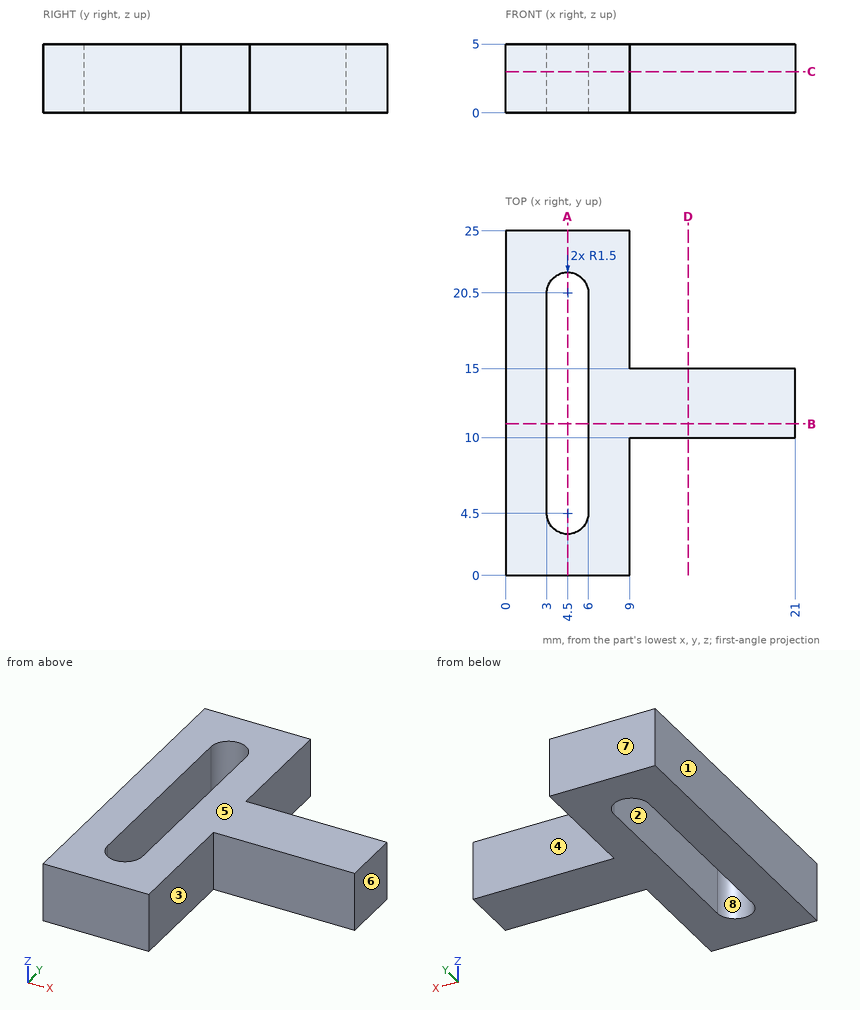
Input: dimensioned drawing with shaded views. Units: mm. Origin: part minimum x, y, z. A direction names the side the tool comes from. Coordinates: 2 decimals unless noted, no trailing zeros. Write each loop counter-clockwise with the first axis right and the second up, starting at its lowest first coordinate (ties: lowest second). Pieces come first, ordered by that corner, then holes. Notation, with made-up numbers: (-14.75, 23) -> (40.25, 23) arc R23 cw to (40.25, 44) -> close; hole circle Ø7 at (-39.5, 81). An arc over 180 degrees is marked (long way). Return JSON: item names as keys, results as strings. Group by question number.
1) Ray query, line 1 along X through (y, z) = (7.5, 1.1); line 2 along X through (y, z) = (12.5, 4.8); line 3 along Y through (x, z) = (10.75, 3.3). Return the intervals inside material, ascending.
2) Section query D-D, the plane x = 13.25. Return loops of the section in (y, z).
3) Section query C-C, the plane z = 3. Return loops of the section in (x, y).
4) Mould query, pull axis X, two halves, no side actions, for the marked faces 6, 7 and 8. Classes: +X half, -X half, draft (parallel to the pull), parting line (faces both ways), or undercut.
5) Section query B-B, the plane y = 11. Return loops of the section in (x, z).
6) Contact query for flat-ended pins moving along their axis: P1, Ø12, axis at x = 12, y = 20, coming from the -Z side; P2, Ø2.5, axis at x = 13.5, z = 3.5, coming from the -Y side; P3, Ø3, axis at x = 16.5, z = 1.5, coming from the +Y side; P4, Ø8, axis at x = 16, y = 20, coming from the -Z side. Output: stop coordinate, or through.
7) Section query A-A, the plane x = 4.5. Return loops of the section in (y, z), plus the area to 3 significant figures.
8) Set-up query: the marked faces 1, 2, 3, 4 and 5. Return all of +Z, -Z, +X, -X, +Y, -Y with unobstructed straight access to the full face (end or side cutting, diameter ignored); none if empty.
From the geometry:
{
 "1": {"line 1": "0 to 3, 6 to 9", "line 2": "0 to 3, 6 to 21", "line 3": "10 to 15"},
 "2": {"outline": "(10, 0) -> (15, 0) -> (15, 5) -> (10, 5) -> close"},
 "3": {"outline": "(0, 0) -> (9, 0) -> (9, 10) -> (21, 10) -> (21, 15) -> (9, 15) -> (9, 25) -> (0, 25) -> close; hole (3, 4.5) arc R1.5 ccw to (6, 4.5) -> (6, 20.5) arc R1.5 ccw to (3, 20.5) -> close"},
 "4": {"face 6": "+X half", "face 7": "draft", "face 8": "undercut"},
 "5": {"outline": "(0, 0) -> (3, 0) -> (3, 5) -> (0, 5) -> close; (6, 0) -> (21, 0) -> (21, 5) -> (6, 5) -> close"},
 "6": {"P1": "z = 0", "P2": "y = 10", "P3": "y = 15", "P4": "through"},
 "7": {"outline": "(0, 0) -> (3, 0) -> (3, 5) -> (0, 5) -> close; (22, 0) -> (25, 0) -> (25, 5) -> (22, 5) -> close", "area": "30.0 mm²"},
 "8": {"face 1": "+Z, -Z, -X, +Y, -Y", "face 2": "+Z, -Z", "face 3": "+Z, -Z, +X, -Y", "face 4": "+Z, -Z, +X, +Y", "face 5": "+Z, +X, -X, +Y, -Y"}
}
